Input: dimensioned drawing with shaded views. Units: mm. Origin: part minimum x, y, z. A direction names the side the tool comes from. Coordinates: 2 decimals unless noted, no trailing zeros. Order: outer loops, then holes, each group sorted by start corner. A loop starts at its lowest first (then second) coordinate and runs counter-clockwise, first axis right, second up. Notation, with made-up numbers: M -38,83 L -15,83 A30 ccw -15,113 Z; hole C 64,59 d9. An arc over 180 degrees is marked long. Use CSV: the item, a comma, the result in double quotes. Start each with the question number.
1. Section query A-A on x = 17.5. Return the cut outline in (y, z), and give its area (3 significant figures).
2. Material intervals for line 1 (Y direction, x = 30, z = 24); line 2 (Z direction, x = 12.5, y = 3); line 3 (Y direction, x = 15, z = 8), sorted ascending.
3. Section query B-B on z = 17.5. Return the cut outline in (x, y).
4. Set-up query: the marked faces 1, 2 and 3. Return all of +Z, -Z, +X, -X, +Y, -Y with unobstructed straight access to the full face (end or side cutting, diameter ignored); none if empty.
5. First-contact query: P1, Ø12, axis at x = 10, z = 11.5, coming from the -Y side; P2, Ø1.5, axis at y = 12, z = 27, coming from the +X side; P3, Ø2, axis at x = 31, z = 29, coming from the -Y side; P4, Ø8, axis at x = 11, z = 8.5, coming from the +Y side. Flat tips, straight axial feed; report the tip coordinate or a pass-through.
6. Section query C-C on y = 15.75. Return the cut outline in (x, z).
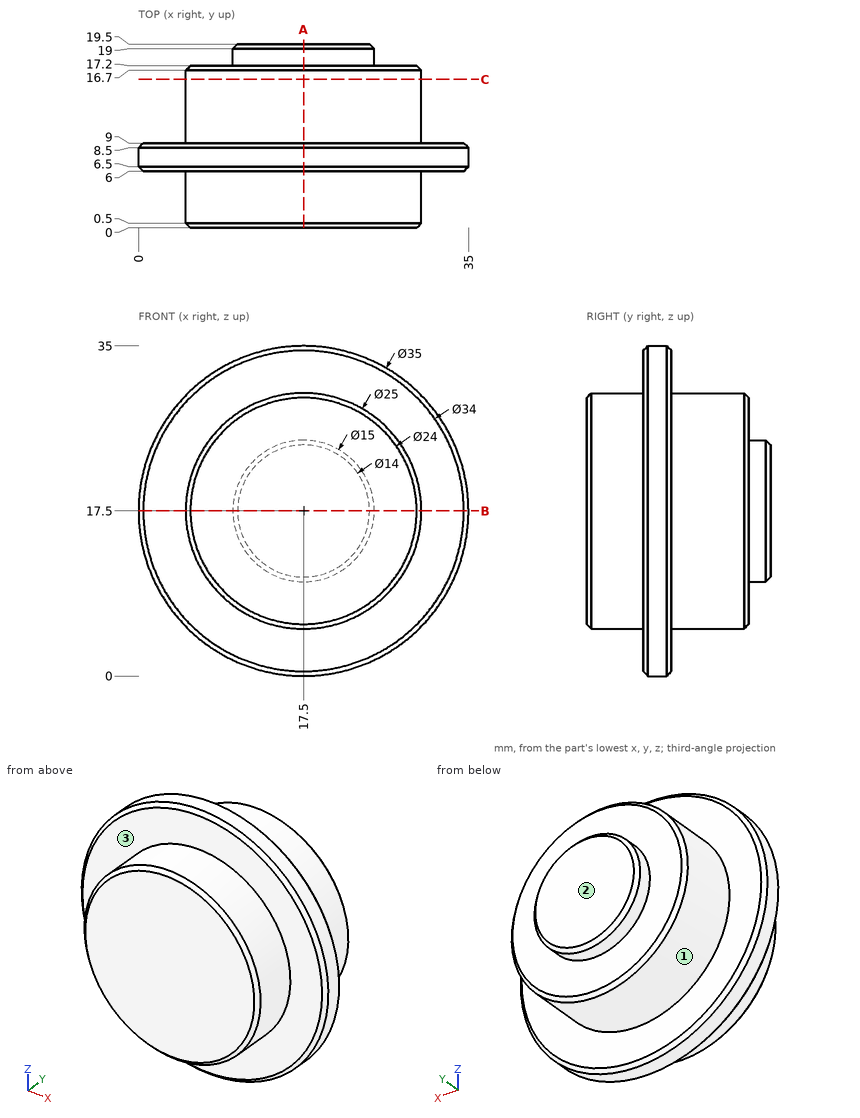
Results list:
1,outline,"M 0,5.5 L 0.5,5 L 6,5 L 6,0.5 L 6.5,0 L 8.5,0 L 9,0.5 L 9,5 L 16.7,5 L 17.2,5.5 L 17.2,10 L 19,10 L 19.5,10.5 L 19.5,24.5 L 19,25 L 17.2,25 L 17.2,29.5 L 16.7,30 L 9,30 L 9,34.5 L 8.5,35 L 6.5,35 L 6,34.5 L 6,30 L 0.5,30 L 0,29.5 Z"
1,area,"493 mm²"
2,line 1,"y = 6 to 9"
2,line 2,"z = 6.04 to 28.96"
2,line 3,"y = 0 to 17.2"
3,outline,"M 0,6.5 L 0.5,6 L 5,6 L 5,0.5 L 5.5,0 L 29.5,0 L 30,0.5 L 30,6 L 34.5,6 L 35,6.5 L 35,8.5 L 34.5,9 L 30,9 L 30,16.7 L 29.5,17.2 L 25,17.2 L 25,19 L 24.5,19.5 L 10.5,19.5 L 10,19 L 10,17.2 L 5.5,17.2 L 5,16.7 L 5,9 L 0.5,9 L 0,8.5 Z"
4,face 1,"+Y"
4,face 2,"+Z, -Z, +X, -X, +Y"
4,face 3,"-Y"
5,P1,"stops at y = 0"
5,P2,"stops at x = 26.43"
5,P3,"stops at y = 6"
5,P4,"stops at y = 19.4"
6,outline,"C 17.5,17.5 d25"
